```python
from build123d import *

# Parameters (mm, degrees)
BOSS_EXTRUDE1_DEPTH = 6
SKETCH3_R           = 3
CUT_EXTRUDE1_DEPTH  = 4
SKETCH9_R           = 2.5
CUT_EXTRUDE2_DEPTH  = 6


with BuildPart() as part:
    # Sketch2 → Boss-Extrude1 (new body)
    with BuildSketch(Plane.XY):
        with BuildLine():
            Line((2.181579686, 9.743947498), (2.181579686, -46.182702418))
            Line((2.181579686, -46.182702418), (-65.818420314, -46.182702418))
            Line((-65.818420314, -46.182702418), (-65.818420314, 9.743947498))
            ThreePointArc((-65.818420314, 9.743947498), (-31.818420314, 43.743947498), (2.181579686, 9.743947498))
        make_face()
    extrude(amount=BOSS_EXTRUDE1_DEPTH)

    # Sketch3 → Cut-Extrude1 (cut)
    with BuildSketch(Plane.XY.offset(6)):
        with Locations((-4.318420314, 9.743947498)):
            Circle(SKETCH3_R)
        with Locations((-31.818420314, -17.756052502)):
            Circle(SKETCH3_R)
        with Locations((-59.318420314, 9.743947498)):
            Circle(SKETCH3_R)
        with Locations((-31.818420314, 37.243947498)):
            Circle(SKETCH3_R)
    extrude(amount=-CUT_EXTRUDE1_DEPTH, mode=Mode.SUBTRACT)

    # Sketch9 → Cut-Extrude2 (cut)
    with BuildSketch(Plane(origin=(0, 0, 0), x_dir=(-1, 0, 0), z_dir=(0, 0, -1))):
        with Locations((45.658538984, 19.210200864)):
            Circle(SKETCH9_R)
        with Locations((17.978301644, 19.210200864)):
            Circle(SKETCH9_R)
        with Locations((31.818420314, -39.753837028)):
            Circle(SKETCH9_R)
    extrude(amount=-CUT_EXTRUDE2_DEPTH, mode=Mode.SUBTRACT)


solid = part.part
```
Read the model definition and answer for the solid it produces. Units are mm, in the model's axes. A direction names the side the tool comes from. Coordinates: 2 decimals unless noted, no trailing zeros. Loops run counter-clockwise (first coordinate to the right, second up) from the corner with the lowest first, then second, coordinate; pieces in that order, holes last.
(1) The part is cut by section A-A (z = 4.75). Determine the outline of the cut face in (x, y).
Solution:
outline: (-65.82, -46.18) - (2.18, -46.18) - (2.18, 9.74) arc R34 ccw to (-65.82, 9.74) - close; hole circle Ø6 at (-59.32, 9.74); hole circle Ø5 at (-45.66, 19.21); hole circle Ø6 at (-31.82, -17.76); hole circle Ø6 at (-31.82, 37.24); hole circle Ø5 at (-31.82, -39.75); hole circle Ø5 at (-17.98, 19.21); hole circle Ø6 at (-4.32, 9.74)
(2) The part is cut by section B-B (x = -46). Determine the outline of the cut face in (y, z), and give its area (3 significant figures).
Solution:
outline: (-46.18, 0) - (16.73, 0) - (16.73, 6) - (-46.18, 6) - close; (21.69, 0) - (40.65, 0) - (40.65, 6) - (21.69, 6) - close
area: 491 mm2
(3) Flat-ended cylindrical pins translate along their axes: pin 1 Ø1 at (y, z) = (32, 2) entering from +X; pin 2 Ø1.8 at (x, y) = (-4.5, 8.5) entering from +Z; pin 3 Ø1 at (x, z) = (-21.5, 4) entering from +Y; pin 4 Ø4.5 at (x, y) = (-45.66, 19.21) entering from -Z. Find the tip coordinate at first contact, or state that the pin passes through.
Solution:
pin 1: stops at x = -5.69
pin 2: stops at z = 2
pin 3: stops at y = 42.3
pin 4: passes through
(4) The part is cut by section D-D (x = -13.5). Determine the outline of the cut face in (y, z), and give its area (3 significant figures).
Solution:
outline: (-46.18, 0) - (38.39, 0) - (38.39, 6) - (-46.18, 6) - close
area: 507 mm2
(5) A tool of negligible diameter and unlimited length cuts with its end or side. For faces 1 (the face through (-65.818, -19, 3)), 2 (the face through (-4, 10, 2)), from which of +Z, -Z, +X, -X, +Y, -Y can it reach the whole face along a straight path? Write none if from no direction.
Solution:
face 1: +Z, -Z, -X, +Y, -Y
face 2: +Z
(6) Consider line 1 along X through (y, z) = (8, 3.8); line 2 along X through (y, z) = (21, 5.05); line 3 along X through (y, z) = (-16, 3.7). Determine where each line is inside the solid, lowest interval first.
Solution:
line 1: x = -65.82 to -61.76, -56.88 to -6.76, -1.88 to 2.18
line 2: x = -63.9 to -47.4, -43.91 to -19.72, -16.23 to 0.26
line 3: x = -65.82 to -34.25, -29.39 to 2.18
(7) The mould has two halves that part along Y. Classify faces 3 (the face through (-31, -46.183, 3)), 4 (the face through (-62.316, 9.876, 4.028)), 5 (the face through (2.182, -18, 3)), 6 (the face through (-32, -18, 2)): released by +Y, released by -Y, zero draft, split by the parting line, or undercut.
Solution:
face 3: released by -Y
face 4: undercut
face 5: zero draft
face 6: undercut
(8) The part is cut by section C-C (y = -19). Determine the outline of the cut face in (x, z).
Solution:
outline: (-65.82, 0) - (2.18, 0) - (2.18, 6) - (-29.09, 6) - (-29.09, 2) - (-34.55, 2) - (-34.55, 6) - (-65.82, 6) - close
